Build history of the part. All positions in model axes, mm. A direction names the side the tool comes from. Round coordinates to 2 decimals unless told otherwise and drop trailing zeros. Write each loop counter-clockwise with the first axis right and the second up, starting at its lowest first coordinate (ties: lowest second). Pieces come first, ordered by that corner, then holes. Notation, with made-up numbers: M 70,18 L 87,18 A20 ccw 87,37 Z; hole C -20,31 d11. An arc over 180 degrees is marked long. Write item = value, one per line. Start each with the question number.
Q1. Probe L1, parallel to X at y = -54, z = 1.15; L2, parallel to Y at x = 48, z = 1.6; L3, parallel to Y at x = 0, z = 1. List the from-to ranges inside material, lowest first.
Q2. Pull direction X, two halves, no side cores. Call faces 3 (the flat face through (-1, 60, 1)), 4 (the flat face through (63, -6, 1)), 5 (the cylindrical face through (-23.74, -39.586, 1.479)): released by +X, released by -X, zero draft, split by the parting line, or undercut.
Q3. Band-saw the part on B-B on x = -48. Write the cut outline in (y, z).
Q4. Band-saw the part on C-C on x = 0. Write the cut outline in (y, z), plus the area to 3 significant figures.
Q5. Band-saw the part on D-D on x = 24. Write the cut outline in (y, z).
Q6. Tool access for faces 1 (the flat face through (-57, 9.6, 2)), 2 (the flat face through (-1, -33, 3)): list every direction of +Z, -Z, +X, -X, +Y, -Y with a clear straight run to the whole face (end or side of a thin tool).
Q7. Band-saw the part on A-A on y = -30. Write the cut outline in (x, z).
```python
from build123d import *

# Parameters (mm, degrees)
SKETCH1_W                    = 126
SKETCH1_H                    = 130
SKETCH1_R                    = 32.5
SKETCH1_W_2                  = 4.9
SKETCH1_H_2                  = 20
BOSS_EXTRUDE1_DEPTH          = 3
SKETCH2_W                    = 2.9
SKETCH2_H                    = 20
CUT_EXTRUDE1_DEPTH           = 3
F_4_0_4_DIAMETER_HOLE1_D     = 4
F_4_0_4_DIAMETER_HOLE1_DEPTH = 10
F_4_0_4_DIAMETER_HOLE1_TIP   = 1.201721238
SKETCH6_R                    = 2.3
CUT_EXTRUDE2_DEPTH           = 3


with BuildPart() as part:
    # Sketch1 → Boss-Extrude1 (new body)
    with BuildSketch(Plane.XY):
        with Locations((0, -5)):
            Rectangle(SKETCH1_W, SKETCH1_H)
        Circle(SKETCH1_R, mode=Mode.SUBTRACT)
        with Locations((-17.5, -54.9)):
            Rectangle(SKETCH1_W_2, SKETCH1_H_2, mode=Mode.SUBTRACT)
        with Locations((17.5, -54.9)):
            Rectangle(SKETCH1_W_2, SKETCH1_H_2, mode=Mode.SUBTRACT)
    extrude(amount=BOSS_EXTRUDE1_DEPTH)

    # Sketch2 → Cut-Extrude1 (cut)
    with BuildSketch(Plane.XY.offset(3)):
        with Locations((-56.5, -0.4)):
            Rectangle(SKETCH2_W, SKETCH2_H)
    cut_extrude1 = extrude(amount=-CUT_EXTRUDE1_DEPTH, mode=Mode.SUBTRACT)

    # Mirror1: Cut-Extrude1 across plane
    add(cut_extrude1.mirror(Plane(origin=(0, 0, 0), x_dir=(0, 0, 1), z_dir=(1, 0, 0))), mode=Mode.SUBTRACT)

    # Ø4.0 (4) Diameter Hole1
    with Locations(Plane.XY.offset(3)):
        with Locations((-24, 41.569219382), (48, 0), (24, 41.569219382), (24, -41.569219382), (-24, -41.569219382), (-48, 0)):
            Hole(F_4_0_4_DIAMETER_HOLE1_D / 2, depth=F_4_0_4_DIAMETER_HOLE1_DEPTH)
            with Locations((0, 0, -(F_4_0_4_DIAMETER_HOLE1_DEPTH + F_4_0_4_DIAMETER_HOLE1_TIP / 2))):  # 118° drill point
                Cone(0, F_4_0_4_DIAMETER_HOLE1_D / 2, F_4_0_4_DIAMETER_HOLE1_TIP, mode=Mode.SUBTRACT)

    # Sketch6 → Cut-Extrude2 (cut)
    with BuildSketch(Plane.XY.offset(3)):
        with Locations((0, -64)):
            Circle(SKETCH6_R)
    extrude(amount=-CUT_EXTRUDE2_DEPTH, mode=Mode.SUBTRACT)


solid = part.part
```
Conclusion:
q1.L1 = -63 to -19.95, -15.05 to 15.05, 19.95 to 63
q1.L2 = -70 to -2, 2 to 60
q1.L3 = -70 to -66.3, -61.7 to -32.5, 32.5 to 60
q2.face_3 = zero draft
q2.face_4 = released by +X
q2.face_5 = undercut
q3.outline = M -70,0 L -2,0 L -2,3 L -70,3 Z; M 2,0 L 60,0 L 60,3 L 2,3 Z
q4.outline = M -70,0 L -66.3,0 L -66.3,3 L -70,3 Z; M -61.7,0 L -32.5,0 L -32.5,3 L -61.7,3 Z; M 32.5,0 L 60,0 L 60,3 L 32.5,3 Z
q4.area = 181 mm^2
q5.outline = M -70,0 L -43.57,0 L -43.57,3 L -70,3 Z; M -39.57,0 L -21.91,0 L -21.91,3 L -39.57,3 Z; M 21.91,0 L 39.57,0 L 39.57,3 L 21.91,3 Z; M 43.57,0 L 60,0 L 60,3 L 43.57,3 Z
q6.face_1 = +Z, -Z
q6.face_2 = +Z, +X, -X, +Y, -Y
q7.outline = M -63,0 L -12.5,0 L -12.5,3 L -63,3 Z; M 12.5,0 L 63,0 L 63,3 L 12.5,3 Z
